Geometry check sheet. Reference: the model listing, model coordinates, mm. A direction names the side the tool comes from. Round coordinates to 2 decimals unless told otherwise and drop trailing zeros. Loops run counter-clockwise (first coordinate to the right, second up) from the corner with the lowest first, then second, coordinate; pieces in that order, holes last. Notation, with made-up numbers: M 73,65.5 L 77,65.5 A16 cw 77,69.5 Z; hole C -12.75,-24 d10. An arc over 180 degrees is marked long. Use one line per item in the form item = value. Start each with the question number.
1. Cross-section at D-D (x = 24). Record the boundary of the cut face in (y, z).
2. Set-up check for faces 1 (the cylindrical face through (-75.8, 30.1, 5.1)), 2 (the flat face through (55, 25, 5)): record each of +Z, -Z, +X, -X, +Y, -Y from which the full face is reachable in a straight line by a thin tool's end or side.
3. Cross-section at A-A (x = 72.5). Record the boundary of the cut face in (y, z).
4. Cross-section at B-B (y = 30). Record the boundary of the cut face in (x, z), then the cut area to 3 significant figures.
5. Go/stop test with a flat-tipped pin: pin 1 (3 mm diameter, centred on x = 6.5, z = 3, fed in from +Y). Record where the tip stops, or that it passes through.
6. Cross-section at C-C (z = 3.5). Record the boundary of the cut face in (x, y).
7. Material ranges on line 1 (Y direction, x = 72.5, z = 5); line 2 (X direction, y = 26, z = 5.25); line 3 (Y direction, x = -20.5, z = 3.75), recorded low to high.
8. Draft check along X on faces 3 (the flat face through (-1, 0, 5)), 4 (the flat face through (72, 50, 5)), 5 (the flat face through (-90, -1, 5)). Enter one of: pulls with the +X half, pulls with the -X half, needs draft (parallel to the pull), parting line crosses it, or undercut.
```python
from build123d import *

# Parameters (mm, degrees)
SKETCH_1_W          = 180
SKETCH_1_H          = 100
EXTRUDE_1_DEPTH     = 10
CUT_EXTRUDE_1_REACH = 105.441
SKETCH_2_W          = 110
SKETCH_2_H          = 100
HOLE_WIZARD_M6_1_D  = 6.6


with BuildPart() as part:
    # 草图1 → 凸台-拉伸1 (new body)
    with BuildSketch(Plane.XY):
        Rectangle(SKETCH_1_W, SKETCH_1_H)
    extrude(amount=EXTRUDE_1_DEPTH)

    # 草图2 → 切除-拉伸1 (cut, up to next)
    with BuildSketch(Plane.XY.offset(10), mode=Mode.PRIVATE) as cut_extrude_1_sk1:
        with Locations((0, 50)):
            Rectangle(SKETCH_2_W, SKETCH_2_H)
    cut_extrude_1_tool1 = extrude(cut_extrude_1_sk1.sketch, amount=-CUT_EXTRUDE_1_REACH, mode=Mode.PRIVATE) & part.part
    add(cut_extrude_1_tool1.solids().sort_by_distance((0, 50, 10))[0], mode=Mode.SUBTRACT)

    # M6 间隙孔1 (through all)
    with Locations(Plane(origin=(0, 0, 0), x_dir=(-1, 0, 0), z_dir=(0, 0, -1))):
        with Locations((-72.5, 30), (72.5, 30)):
            Hole(HOLE_WIZARD_M6_1_D / 2)


solid = part.part
```
Reported:
q1.outline = M -50,0 L 0,0 L 0,10 L -50,10 Z
q2.face_1 = +Z, -Z
q2.face_2 = +Z, -Z, +Y
q3.outline = M -50,0 L 26.7,0 L 26.7,10 L -50,10 Z; M 33.3,0 L 50,0 L 50,10 L 33.3,10 Z
q4.outline = M -90,0 L -75.8,0 L -75.8,10 L -90,10 Z; M -69.2,0 L -55,0 L -55,10 L -69.2,10 Z; M 55,0 L 69.2,0 L 69.2,10 L 55,10 Z; M 75.8,0 L 90,0 L 90,10 L 75.8,10 Z
q4.area = 568 mm²
q5.pin_1 = 0
q6.outline = M -90,-50 L 90,-50 L 90,50 L 55,50 L 55,0 L -55,0 L -55,50 L -90,50 Z; hole C -72.5,30 d6.6; hole C 72.5,30 d6.6
q7.line_1 = -50 to 26.7, 33.3 to 50
q7.line_2 = -90 to -55, 55 to 90
q7.line_3 = -50 to 0
q8.face_3 = undercut
q8.face_4 = needs draft
q8.face_5 = pulls with the -X half
